Geometry: final body of the model. Coordinates: model frame, mm. Face numbers are marked on the shaded views. A direction names the side the tool comes from. Coordinates: 2 decimals unless noted, no trailing zeros. Write each loop counter-clockwise with the first axis right and the second up, starting at its lowest first coordinate (ties: lowest second). Pieces come first, ordered by that corner, then holes. Notation, with made-up numbers: (7.25, -39) -> (48.25, -39) arc R17 ccw to (48.25, -16) -> close; hole circle Ø4 at (7.5, 30.25). An arc over 180 degrees is marked (long way). One line per item, written item: value.
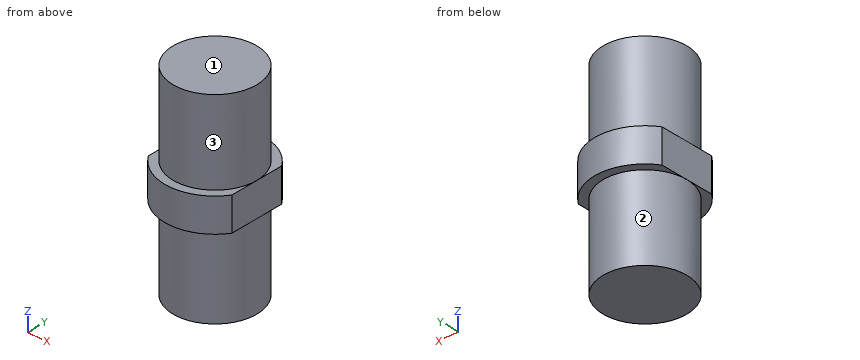
```python
from build123d import *

# Parameters (mm, degrees)
BOSS_EXTRUDE1_DEPTH = 4
SKETCH2_W           = 5
SKETCH2_H           = 10
SKETCH3_W           = 5
SKETCH3_H           = 10


with BuildPart() as part:
    # Sketch1 → Boss-Extrude1 (new body)
    with BuildSketch(Plane.XY.offset(4)):
        with BuildLine():
            Line((5, -3.31662479), (5, 3.31662479))
            ThreePointArc((5, 3.31662479), (0, 6), (-5, 3.31662479))
            Line((-5, 3.31662479), (-5, -3.31662479))
            ThreePointArc((-5, -3.31662479), (0, -6), (5, -3.31662479))
        make_face()
    extrude(amount=-BOSS_EXTRUDE1_DEPTH)

    # Sketch2 → Revolve1 (revolve)
    with BuildSketch(Plane(origin=(0, 0, 0), x_dir=(1, 0, 0), z_dir=(0, 1, 0))):
        with Locations((2.5, -9)):
            Rectangle(SKETCH2_W, SKETCH2_H)
    revolve(axis=Axis((0, 0, 4), (0, 0, 1)))

    # Sketch3 → Revolve2 (revolve)
    with BuildSketch(Plane.XZ, mode=Mode.PRIVATE) as revolve2_sk:
        with Locations((2.5, -5)):
            Rectangle(SKETCH3_W, SKETCH3_H)
    revolve(revolve2_sk.sketch.rotate(Axis((0, 0, 0), (0, 0, -1)), 180), axis=Axis((0, 0, 0), (0, 0, -1)))


solid = part.part
```
(1) Line query: line 1 (X direction, y = 5, z = 2); line 2 (Z direction, x = -3.25, y = -5); line 3 (Y direction, x = 0.25, z = 12.75). Output: solid intervals per line, ascending. Write a range as [from, to].
Responses:
line 1: x = [-3.32, 3.32]
line 2: z = [0, 4]
line 3: y = [-4.99, 4.99]
(2) Section A-A (x = 2). Return the cut outline in (y, z), then the cut area to 3 significant figures.
Responses:
outline: (-5.66, 0) -> (-4.58, 0) -> (-4.58, -10) -> (4.58, -10) -> (4.58, 0) -> (5.66, 0) -> (5.66, 4) -> (4.58, 4) -> (4.58, 14) -> (-4.58, 14) -> (-4.58, 4) -> (-5.66, 4) -> close
area: 229 mm2
(3) Reachability of the marked faces 1, 2 and 3 from +Z, -Z, +X, -X, +Y, -Y: full face, straight path, thin tool, end or side. Return the list, or none.
Responses:
face 1: +Z, +X, -X, +Y, -Y
face 2: -Z
face 3: +Z
(4) Section C-C (x = 4.25). Return the cut outline in (y, z).
Responses:
outline: (-4.24, 0) -> (-2.63, 0) -> (-2.63, -10) -> (2.63, -10) -> (2.63, 0) -> (4.24, 0) -> (4.24, 4) -> (2.63, 4) -> (2.63, 14) -> (-2.63, 14) -> (-2.63, 4) -> (-4.24, 4) -> close
(5) Section D-D (z = 1.75). Return the cut outline in (x, y), then the cut area to 3 significant figures.
Responses:
outline: (-5, -3.32) arc R6 ccw to (5, -3.32) -> (5, 3.32) arc R6 ccw to (-5, 3.32) -> close
area: 104 mm2
(6) Section B-B (z = 4.25). Return the cut outline in (x, y).
Responses:
outline: circle Ø10 at (0, 0)
